from build123d import *

# Parameters (mm, degrees)
SKETCH1_W           = 46
SKETCH1_H           = 65
BOSS_EXTRUDE1_DEPTH = 8
SKETCH2_R           = 2.75
CUT_EXTRUDE1_DEPTH  = 18
CHAMFER1_SIZE       = 10
SKETCH3_R           = 2.75
CUT_EXTRUDE2_DEPTH  = 10
SKETCH4_W           = 18
SKETCH4_H           = 45
CUT_EXTRUDE3_DEPTH  = 10
SKETCH5_R           = 2.75
BOSS_EXTRUDE2_DEPTH = 2
FILLET1_R           = 2
CHAMFER2_SIZE       = 3


with BuildPart() as part:
    # Sketch1 → Boss-Extrude1 (new body)
    with BuildSketch(Plane.XY):
        with Locations((-23, 32.5)):
            Rectangle(SKETCH1_W, SKETCH1_H)
    extrude(amount=BOSS_EXTRUDE1_DEPTH)

    # Sketch2 → Cut-Extrude1 (cut)
    with BuildSketch(Plane.XY.offset(8)):
        with Locations((-10.5, 10)):
            Circle(SKETCH2_R)
    extrude(amount=-CUT_EXTRUDE1_DEPTH, mode=Mode.SUBTRACT)

    # Chamfer1
    chamfer1_edges = [part.edges().sort_by_distance(p)[0] for p in [
        (-46, 0, 4),
    ]]
    chamfer(chamfer1_edges, length=CHAMFER1_SIZE)

    # Sketch3 → Cut-Extrude2 (cut)
    with BuildSketch(Plane.XY.offset(8)):
        with Locations((-32, 55)):
            Circle(SKETCH3_R)
        with Locations((-32, 30)):
            Circle(SKETCH3_R)
    extrude(amount=-CUT_EXTRUDE2_DEPTH, mode=Mode.SUBTRACT)

    # Sketch4 → Cut-Extrude3 (cut)
    with BuildSketch(Plane.XY.offset(8)):
        with Locations((-9, 42.5)):
            Rectangle(SKETCH4_W, SKETCH4_H)
    extrude(amount=-CUT_EXTRUDE3_DEPTH, mode=Mode.SUBTRACT)

    # Sketch5 → Boss-Extrude2 (add)
    with BuildSketch(Plane(origin=(0, 0, 0), x_dir=(-1, 0, 0), z_dir=(0, 0, -1))):
        Polygon((0, 20), (46, 20), (46, 10), (36, 0), (0, 0), align=None)
        with Locations(Location((10.5, 10, 0), (0, 0, 180))):
            Circle(SKETCH5_R, mode=Mode.SUBTRACT)
    extrude(amount=BOSS_EXTRUDE2_DEPTH)

    # Fillet1
    fillet1_edges = [part.edges().sort_by_distance(p)[0] for p in [
        (-18, 20, 4),
    ]]
    fillet(fillet1_edges, radius=FILLET1_R)

    # Chamfer2
    chamfer2_edges = [part.edges().sort_by_distance(p)[0] for p in [
        (0, 0, 3),
        (0, 20, 3),
        (-18, 65, 4),
        (-46, 65, 4),
    ]]
    chamfer(chamfer2_edges, length=CHAMFER2_SIZE)


solid = part.part
For this review, take the finished solid that the model builds, in its own axes (mm). A direction names the side the tool comes from. Round coordinates to 2 decimals unless told otherwise and drop trailing zeros. Loops run counter-clockwise (first coordinate to the right, second up) from the corner with the lowest first, then second, coordinate; pieces in that order, holes last. Notation, with made-up numbers: (-8.75, -3) - (34.25, -3) arc R27 ccw to (34.25, 25) - close; hole circle Ø9 at (-12.5, -40). An arc over 180 degrees is marked (long way). Use one line per item in the form item = value.
Item 1: Tool access review of faces 5 (the flat face through (-15, 20, 2)), 6 (the flat face through (-18, 42, 4)), 7 (the flat face through (-45, 63, 4)): name each direction out of +Z, -Z, +X, -X, +Y, -Y from which nothing blocks a thin tool from reaching the whole face with its end or side.
Answers:
face_5 = -Z, +X, +Y
face_6 = +Z, -Z, +X, +Y
face_7 = +Z, -Z, -X, +Y
Item 2: Consider section B-B on x = -32. Write out the cut boundary in (y, z), then the cut area to 3 significant figures.
Answers:
outline = (0, -2) - (20, -2) - (20, 0) - (27.25, 0) - (27.25, 8) - (0, 8) - close; (32.75, 0) - (52.25, 0) - (52.25, 8) - (32.75, 8) - close; (57.75, 0) - (65, 0) - (65, 8) - (57.75, 8) - close
area = 472 mm^2
Item 3: Consider section D-D on x = -10.5. Write out the cut boundary in (y, z), then the cut area to 3 significant figures.
Answers:
outline = (0, -2) - (7.25, -2) - (7.25, 8) - (0, 8) - close; (12.75, -2) - (20, -2) - (20, 8) - (12.75, 8) - close
area = 145 mm^2
Item 4: Clearance check with flat-ended pins moving along their axes: P1, Ø9, axis at x = -36.5, y = 41.5, coming from the -Z side; P2, Ø4.5, axis at x = -32, y = 55, coming from the -Z side. State where each tip first meets the part, or that it passes through.
Answers:
P1 = 0
P2 = through
Item 5: Mouldability with a two-part tool opening along Y and no side actions: class faces 1 (the flat face through (-35, 43, 0)), 2 (the flat face through (-20, 64, 4)), 3 (the cylindrical face through (-34.027, 31.859, 4.056)), 4 (the flat face through (-41, 5, 3)) as +Y half, -Y half, draft (parallel to the pull), parting line (faces both ways), or undercut.
Answers:
face_1 = draft
face_2 = +Y half
face_3 = undercut
face_4 = -Y half
Item 6: Consider section C-C on z = 5. Write out the cut boundary in (x, y).
Answers:
outline = (-46, 10) - (-36, 0) - (-3, 0) - (0, 3) - (0, 17) - (-3, 20) - (-16, 20) arc R2 cw to (-18, 22) - (-18, 62) - (-21, 65) - (-43, 65) - (-46, 62) - close; hole circle Ø5.5 at (-32, 30); hole circle Ø5.5 at (-32, 55); hole circle Ø5.5 at (-10.5, 10)
Item 7: For line 1 (Y direction, x = -32, z = 2.5); line 2 (X direction, y = 10, z = 2.5); line 3 (Y direction, x = -29.5, z = 1.75), list the stretches that pass through material, from the lowest coordinate up.
Answers:
line_1 = 0 to 27.25, 32.75 to 52.25, 57.75 to 65
line_2 = -46 to -13.25, -7.75 to 0
line_3 = 0 to 28.85, 31.15 to 53.85, 56.15 to 65
Item 8: Consider section A-A on y = 55. Write out the cut boundary in (x, z), then the cut area to 3 significant figures.
Answers:
outline = (-46, 0) - (-34.75, 0) - (-34.75, 8) - (-46, 8) - close; (-29.25, 0) - (-18, 0) - (-18, 8) - (-29.25, 8) - close
area = 180 mm^2
